Read the model definition and answer for the solid it produces. Units are mm, in the model's axes. Coordinates: 2 decimals unless noted, no trailing zeros. Loops run counter-clockwise (first coordinate to the right, second up) from the corner with the lowest first, then second, coordinate; pieces in that order, holes last. Notation, with made-up numbers: (17.5, -29.75) - (50.5, -29.75) arc R13 cw to (50.5, -8.75) - close; hole circle Ø7 at (87, 16.5). An arc over 180 degrees is marked (long way). One line per item, written item: value. Start each with the question number.
from build123d import *

# Parameters (mm, degrees)
SKETCH_1_W          = 540
SKETCH_1_H          = 540
EXTRUDE_1_DEPTH     = 1
SKETCH_2_R          = 9
CUT_EXTRUDE_1_DEPTH = 382.838971295
SKETCH_3_R          = 20
CUT_EXTRUDE_2_DEPTH = 382.838971295
SKETCH_4_R          = 25
CUT_EXTRUDE_3_DEPTH = 10
SKETCH_5_R          = 17.5
CUT_EXTRUDE_4_DEPTH = 382.838971295


with BuildPart() as part:
    # 草图1 → 凸台-拉伸1 (new body)
    with BuildSketch(Plane.XY):
        Rectangle(SKETCH_1_W, SKETCH_1_H)
    extrude(amount=EXTRUDE_1_DEPTH)

    # 草图2 → 切除-拉伸1 (cut, through all)
    with BuildSketch(Plane(origin=(0, 0, 0), x_dir=(-1, 0, 0), z_dir=(0, 0, -1))):
        with Locations((250, -255)):
            Circle(SKETCH_2_R)
        with Locations((-250, -255)):
            Circle(SKETCH_2_R)
        with Locations((250, 255)):
            Circle(SKETCH_2_R)
        with Locations((-250, 255)):
            Circle(SKETCH_2_R)
    extrude(amount=-CUT_EXTRUDE_1_DEPTH, mode=Mode.SUBTRACT)

    # 草图3 → 切除-拉伸2 (cut, through all)
    with BuildSketch(Plane.XY.offset(1)):
        with Locations((-210, 0)):
            Circle(SKETCH_3_R)
        with Locations((210, 0)):
            Circle(SKETCH_3_R)
    extrude(amount=-CUT_EXTRUDE_2_DEPTH, mode=Mode.SUBTRACT)

    # 草图4 → 切除-拉伸3 (cut)
    with BuildSketch(Plane.XY.offset(1)):
        Circle(SKETCH_4_R)
    extrude(amount=-CUT_EXTRUDE_3_DEPTH, mode=Mode.SUBTRACT)

    # 草图5 → 切除-拉伸4 (cut, through all)
    with BuildSketch(Plane(origin=(0, 0, 0), x_dir=(-1, 0, 0), z_dir=(0, 0, -1))):
        with Locations((0, -190)):
            Circle(SKETCH_5_R)
        with Locations((0, 210)):
            Circle(SKETCH_5_R)
    extrude(amount=-CUT_EXTRUDE_4_DEPTH, mode=Mode.SUBTRACT)


solid = part.part
1) Section D-D, the plane y = 210 is taken. Determine the outline of the cut face in (x, z).
2) Section B-B, the plane y = 0 is taken. Determine the outline of the cut face in (x, z), and give its area (3 significant figures).
3) Straight lines are drawn through the part: L1, parallel to Y at x = 210, z = 0.45; L2, parallel to Y at x = -250, z = 0.8; L3, parallel to Y at x = 0, z = 0.5. For each, find the intervals that lie inside material, in ascending order.
4) Section C-C, the plane z = 0.25 is taken. State how many separate pieces and enclosed holes the cut face has, and give its area (3 significant figures).
5) Determine the mould class of faces 1 (the flat face through (-4, 64, 0)), 2 (the cylindrical face through (251.951, 246.214, 0.493)) for opening direction Y: released by +Y, released by -Y, zero draft, split by the parting line, or undercut.
6) Section A-A, the plane x = 210 is taken. Determine the outline of the cut face in (y, z).
Answer below:
1. outline: (-270, 0) - (-17.5, 0) - (-17.5, 1) - (-270, 1) - close; (17.5, 0) - (270, 0) - (270, 1) - (17.5, 1) - close
2. outline: (-270, 0) - (-230, 0) - (-230, 1) - (-270, 1) - close; (-190, 0) - (-25, 0) - (-25, 1) - (-190, 1) - close; (25, 0) - (190, 0) - (190, 1) - (25, 1) - close; (230, 0) - (270, 0) - (270, 1) - (230, 1) - close
2. area: 410 mm2
3. L1: -270 to -20, 20 to 270
3. L2: -270 to -264, -246 to 246, 264 to 270
3. L3: -270 to -207.5, -172.5 to -25, 25 to 192.5, 227.5 to 270
4. separate pieces: 1
4. enclosed holes: 9
4. area: 284,000 mm2
5. face 1: zero draft
5. face 2: undercut
6. outline: (-270, 0) - (-20, 0) - (-20, 1) - (-270, 1) - close; (20, 0) - (270, 0) - (270, 1) - (20, 1) - close
